Source: CAD feature listing. Evaluate the final solid. Frame: model axes, mm. A direction names the side the tool comes from. Give positions to 0.01 mm unless a question says otherwise; leave off trailing zeros. Loops run counter-clockwise (first coordinate to the right, second up) from the corner with the lowest first, then second, coordinate; pieces in that order, holes last. Notation, with made-up numbers: (0, 73.5) -> (25, 73.5) arc R9 cw to (25, 85.5) -> close; hole circle Ø8 at (-33.75, 15). An arc over 180 degrees is marked (long way). Answer as a JSON object with one key per item and string values. Group by question number.
from build123d import *

# Parameters (mm, degrees)
RING_HUB_PROFILE_R       = 25
RING_HUB_DEPTH           = 43
FLANGE_PROFILE_3_HOLES_R = 4
TRIANGULAR_FLANGE_DEPTH  = 7
BOSS_BORE_PROFILE_R      = 10
BOSS_BORE_DEPTH          = 13
FLANGE_START             = 3
FLANGE_BOSS_PROFILE_R    = 16
FLANGE_BOSS_PROFILE_R_2  = 10
FLANGE_BOSS_32_DEPTH     = 3
HUB_SLIT_PROFILE_R       = 9
HUB_SLIT_CUT_DEPTH       = 67.5


with BuildPart() as part:
    # Ring Hub Profile → Ring Hub (new, symmetric)
    with BuildSketch(Plane.XY):
        with BuildLine():
            Line((0, 34), (60, 34))
            Line((60, 34), (60, 25))
            Line((60, 25), (33.481338086, 25))
            ThreePointArc((33.481338086, 25), (29.132745622, 22.467740584), (29.188858844, 17.435897436))
            ThreePointArc((29.188858844, 17.435897436), (-16.780635971, -29.570428749), (0, 34))
        make_face()
        Circle(RING_HUB_PROFILE_R, mode=Mode.SUBTRACT)
    extrude(amount=RING_HUB_DEPTH, both=True)

    # Flange Profile 3 Holes → Triangular Flange (add, symmetric)
    with BuildSketch(Plane(origin=(0, 29.5, 0), x_dir=(1, 0, 0), z_dir=(0, 1, 0))):
        with BuildLine():
            Line((63.910945409, 41.975055486), (118.910945409, 5.975055486))
            ThreePointArc((118.910945409, 5.975055486), (122.141203123, 0), (118.910945409, -5.975055486))
            Line((118.910945409, -5.975055486), (63.910945409, -41.975055486))
            ThreePointArc((63.910945409, -41.975055486), (56.603831094, -42.281943872), (52.858796877, -36))
            Line((52.858796877, -36), (52.858796877, 36))
            ThreePointArc((52.858796877, 36), (56.603831094, 42.281943872), (63.910945409, 41.975055486))
        make_face()
        with Locations(Location((60, 36, 0), (0, 0, 270))):
            Circle(FLANGE_PROFILE_3_HOLES_R, mode=Mode.SUBTRACT)
        with Locations(Location((60, -36, 0), (0, 0, 270))):
            Circle(FLANGE_PROFILE_3_HOLES_R, mode=Mode.SUBTRACT)
        with Locations(Location((115, 0, 0), (0, 0, 270))):
            Circle(FLANGE_PROFILE_3_HOLES_R, mode=Mode.SUBTRACT)
    extrude(amount=TRIANGULAR_FLANGE_DEPTH, both=True)

    # Boss Bore Profile → Boss Bore (cut, symmetric)
    with BuildSketch(Plane(origin=(0, 29.5, 0), x_dir=(1, 0, 0), z_dir=(0, 1, 0))):
        with Locations(Location((75, 0, 0), (0, 0, 270))):
            Circle(BOSS_BORE_PROFILE_R)
    extrude(amount=BOSS_BORE_DEPTH, both=True, mode=Mode.SUBTRACT)

    # Flange Boss Profile → Flange Boss Ø32 (add)
    with BuildSketch(Plane(origin=(0, 36.5, 0), x_dir=(1, 0, 0), z_dir=(0, 1, 0)).offset(FLANGE_START)):
        with Locations(Location((75, 0, 0), (0, 0, 270))):
            Circle(FLANGE_BOSS_PROFILE_R)
        with Locations(Location((75, 0, 0), (0, 0, 270))):
            Circle(FLANGE_BOSS_PROFILE_R_2, mode=Mode.SUBTRACT)
    extrude(amount=-FLANGE_BOSS_32_DEPTH)

    # Hub Revolve Profile → Hub Revolved Feature (revolve)
    with BuildSketch(Plane.XY):
        with BuildLine():
            Line((-32.526911935, -9.899494937), (-62.805081277, -40.177664279))
            Line((-62.805081277, -40.177664279), (-57.855333809, -45.127411748))
            Line((-57.855333809, -45.127411748), (-29.548007269, -16.820085208))
            ThreePointArc((-29.548007269, -16.820085208), (-31.229754097, -13.442561476), (-32.526911935, -9.899494937))
        make_face()
    revolve(axis=Axis((0, 0, 0), (-0.7071067811865461, -0.707106781186549, 0)))

    # Hub Slit Profile → Hub Slit Cut (cut, symmetric)
    with BuildSketch(Plane(origin=(-51.491372778, -51.491372778, 0), x_dir=(0, 0, 1), z_dir=(-0.7071067811865462, -0.7071067811865489, 0))):
        with Locations(Location((0, 0, 0), (0, 0, 90))):
            Circle(HUB_SLIT_PROFILE_R)
    extrude(amount=HUB_SLIT_CUT_DEPTH, both=True, mode=Mode.SUBTRACT)


solid = part.part
(1) Section query B-B on x = 75. Return the cut outline in (y, z).
(2) Material intervals for line 1 (Y direction, x = 0, z = -22); line 2 (Y direction, x = 37, z = 37.5); line 3 (Z direction, x = 10, y = -25), sorted ascending. Write a range as from..to.
(3) Access query for faces 4 (the face through (23, 13, 43)), 5 (the face through (63.966, 29.402, 35.479)), 6 (the face through (58, 34, -36)), 7 (the face through (60, 30, -36)). Directions: +Z, -Z, +X, -X, +Y, -Y. A direction counts if a zero-diameter tool reaches every point of the face in a straight line with its end or side. Return the directions, or none.
(4) Section query D-D on z = 29.5. Return the cut outline in (x, y).
(5) Section query C-C on y = 30.5. Return the cut outline in (x, z), plus the area to 3 significant figures.
(6) Section query A-A on z = 20.5. Return the cut outline in (x, y).
(7) Mould query, pull axis Z, two halves, no side actions, for faces 1 (the face through (23, 13, -43)), 2 (the face through (122.14, 29.6, -0.1)), 3 (the face through (118.966, 29.402, -0.521)). Classes: pulls with the +Z half, pulls with the -Z half, needs draft (parallel to the pull), parting line crosses it, or undercut.
(8) First-contact query: pin 1 (2 mm diameter, centred on x = 86, z = -28.5, fed in from +Y); pin 2 (4 mm diameter, centred on x = 22, z = 12, fed in from -Y); pin 3 (10 mm diameter, centred on y = 12, z = -32.5, fed in from -X). Flat tips, straight axial feed; report the tip coordinate or a pass-through.
Result:
{
 "1": {"outline": "(22.5, -34.72) -> (36.5, -34.72) -> (36.5, -16) -> (39.5, -16) -> (39.5, -10) -> (22.5, -10) -> close; (22.5, 10) -> (39.5, 10) -> (39.5, 16) -> (36.5, 16) -> (36.5, 34.72) -> (22.5, 34.72) -> close"},
 "2": {"line 1": "-34..-25, 25..34", "line 2": "25..34", "line 3": "-43..43"},
 "3": {"face 4": "+Z, -X, +Y, -Y", "face 5": "none", "face 6": "+Y", "face 7": "+Y, -Y"},
 "4": {"outline": "(0, 34) arc R34 ccw (long way) to (29.19, 17.44) arc R5 cw to (33.48, 25) -> (52.86, 25) -> (52.86, 22.5) -> (82.97, 22.5) -> (82.97, 36.5) -> (52.86, 36.5) -> (52.86, 34) -> close; hole circle Ø50 at (0, 0)"},
 "5": {"outline": "(-15.02, -43) -> (58.59, -43) arc R7.14 ccw to (63.91, -41.98) -> (118.91, -5.98) arc R7.14 ccw to (118.91, 5.98) -> (63.91, 41.98) arc R7.14 ccw to (58.59, 43) -> (-15.02, 43) -> close; hole (60, -40) arc R4 ccw to (60, -32) -> close; hole (60, 32) arc R4 ccw to (60, 40) -> close; hole circle Ø20 at (75, 0); hole circle Ø8 at (115, 0)", "area": "9,040 mm²"},
 "6": {"outline": "(0, 34) arc R34 ccw (long way) to (29.19, 17.44) arc R5 cw to (33.48, 25) -> (52.86, 25) -> (52.86, 22.5) -> (96.72, 22.5) -> (96.72, 36.5) -> (52.86, 36.5) -> (52.86, 34) -> close; hole circle Ø50 at (0, 0)"},
 "7": {"face 1": "pulls with the -Z half", "face 2": "parting line crosses it", "face 3": "undercut"},
 "8": {"pin 1": "y = 36.5", "pin 2": "y = -27.5", "pin 3": "x = -33.27"}
}
